Check sheet for the modelled part. Datum: model origin and axes. Units: mm. A direction names the side the tool comes from. Coordinates: 2 decimals unless noted, no trailing zeros. Loops run counter-clockwise (first coordinate to the right, second up) from the corner with the lowest first, then second, coordinate; pieces in that order, holes last. Notation, with made-up numbers: (69, 65.25) - (84, 65.25) arc R34 cw to (84, 96.25) - close; hole circle Ø8 at (70, -29.5). An arc over 180 degrees is marked (long way). Write each question's results on one line, items separated by ' | '. Start each with the question number.
1. Cross-section at B-B (z = 11). Record the cut outline in (x, y).
2. Tool access check on faces 4 (the face through (-2, 15, -31)), 5 (the face through (1, 46, -26)), 6 (the face through (-101, 32, 5)). Record the directions out of +Z, -Z, +X, -X, +Y, -Y that give a thin tool (end or side, any length) a straight path to the whole face; none if there is none.
3. Cross-section at C-C (y = 12). Record the cut outline in (x, z).
4. Draft check along X on faces 1 (the face through (-131, 5, 0)), 2 (the face through (20.24, 20.5, -26.07)), 3 (the face through (-41.17, 44.574, -26.07)). Enter one of: released by +X, released by -X, zero draft, split by the parting line, or undercut.
5. Cross-section at D-D (x = 26). Record the cut outline in (y, z).
6. Cross-section at A-A (x = 62). Record the cut outline in (y, z), and give its area (3 significant figures).
7. Gauge pin test, flat ends, axial feed: P1, Ø1.5, axis at x = -11.5, y = 48, coming from the +Z side; P2, Ø11, axis at y = 30.5, z = -26.5, coming from the -X side; P3, Ø11, axis at y = 29.5, z = -26.5, coming from the +X side. Record the tip position at first contact, or that the pin passes through.
8. Thickness scan on line 1 (Y direction, x = 37, z = 15); line 2 (X direction, y = 32, z = -24); line 3 (X direction, y = 55.5, z = -13). Record the ranges inside material, lowest first. Write a range as [from, to].
```python
from build123d import *

# Parameters (mm, degrees)
SKETCH_1_W          = 300
SKETCH_1_H          = 62
EXTRUDE_1_DEPTH     = 5
SKETCH_2_W          = 298.120909486
SKETCH_2_H          = 12
CUT_EXTRUDE_1_DEPTH = 1.5
SKETCH_3_W          = 15
SKETCH_3_H          = 62
SKETCH_3_W_2        = 14
CUT_EXTRUDE_2_DEPTH = 1.5
EXTRUDE_2_DEPTH     = 55
SKETCH_5_W          = 222
SKETCH_5_H          = 62
EXTRUDE_3_DEPTH     = 8
CUT_EXTRUDE_3_REACH = 174.708
SKETCH_6_W          = 41.333333333
SKETCH_6_H          = 27
SKETCH_6_W_2        = 41.333333334
FILLET_1_R          = 5


with BuildPart() as part:
    # 草图1 → 凸台-拉伸1 (new, symmetric)
    with BuildSketch(Plane(origin=(0, 0, 0), x_dir=(1, 0, 0), z_dir=(0, 1, 0))):
        Rectangle(SKETCH_1_W, SKETCH_1_H)
    extrude(amount=EXTRUDE_1_DEPTH, both=True)

    # 草图2 → 切除-拉伸1 (cut)
    with BuildSketch(Plane.XZ.offset(5)):
        with Locations((0.939545257, 25)):
            Rectangle(SKETCH_2_W, SKETCH_2_H)
    extrude(amount=-CUT_EXTRUDE_1_DEPTH, mode=Mode.SUBTRACT)

    # 草图3 → 切除-拉伸2 (cut)
    with BuildSketch(Plane.XZ.offset(5)):
        with Locations((-142.5, 0)):
            Rectangle(SKETCH_3_W, SKETCH_3_H)
        with Locations((143, 0)):
            Rectangle(SKETCH_3_W_2, SKETCH_3_H)
    extrude(amount=-CUT_EXTRUDE_2_DEPTH, mode=Mode.SUBTRACT)

    # 草图4 → 凸台-拉伸2 (add)
    with BuildSketch(Plane(origin=(0, 5, 0), x_dir=(1, 0, 0), z_dir=(0, 1, 0))):
        Polygon((-111, -31), (-111, 31), (111, 31), (111, -31), (103, -31), (103, 21), (-101, 21), (-101, -31), align=None)
    extrude(amount=EXTRUDE_2_DEPTH)

    # 草图5 → 凸台-拉伸3 (add)
    with BuildSketch(Plane(origin=(0, 60, 0), x_dir=(1, 0, 0), z_dir=(0, 1, 0))):
        Rectangle(SKETCH_5_W, SKETCH_5_H)
    extrude(amount=EXTRUDE_3_DEPTH)

    # 草图6 → 切除-拉伸3 (cut, up to next)
    with BuildSketch(Plane.XY.offset(-21), mode=Mode.PRIVATE) as cut_extrude_3_sk1:
        with Locations((-60.333333334, 32.5)):
            Rectangle(SKETCH_6_W, SKETCH_6_H)
    cut_extrude_3_tool1 = extrude(cut_extrude_3_sk1.sketch, amount=-CUT_EXTRUDE_3_REACH, mode=Mode.PRIVATE) & part.part
    # 草图6 → 切除-拉伸3 (cut, up to next)
    with BuildSketch(Plane.XY.offset(-21), mode=Mode.PRIVATE) as cut_extrude_3_sk2:
        with Locations((62.333333334, 32.5)):
            Rectangle(SKETCH_6_W, SKETCH_6_H)
    cut_extrude_3_tool2 = extrude(cut_extrude_3_sk2.sketch, amount=-CUT_EXTRUDE_3_REACH, mode=Mode.PRIVATE) & part.part
    # 草图6 → 切除-拉伸3 (cut, up to next)
    with BuildSketch(Plane.XY.offset(-21), mode=Mode.PRIVATE) as cut_extrude_3_sk3:
        with Locations((1, 32.5)):
            Rectangle(SKETCH_6_W_2, SKETCH_6_H)
    cut_extrude_3_tool3 = extrude(cut_extrude_3_sk3.sketch, amount=-CUT_EXTRUDE_3_REACH, mode=Mode.PRIVATE) & part.part
    add(cut_extrude_3_tool1.solids().sort_by_distance((-60.333333, 32.5, -21))[0], mode=Mode.SUBTRACT)
    add(cut_extrude_3_tool2.solids().sort_by_distance((62.333333, 32.5, -21))[0], mode=Mode.SUBTRACT)
    add(cut_extrude_3_tool3.solids().sort_by_distance((1, 32.5, -21))[0], mode=Mode.SUBTRACT)

    # 圆角1
    fillet_1_edges = [part.edges().sort_by_distance(p)[0] for p in [
        (-39.666666667, 46, -26),
        (-39.666666667, 19, -26),
        (-81, 19, -26),
        (-81, 46, -26),
        (83, 46, -26),
        (83, 19, -26),
        (41.666666667, 19, -26),
        (41.666666667, 46, -26),
        (21.666666667, 46, -26),
        (21.666666667, 19, -26),
        (-19.666666667, 19, -26),
        (-19.666666667, 46, -26),
    ]]
    fillet(fillet_1_edges, radius=FILLET_1_R)


solid = part.part
```
Established:
1) outline: (-150, -3.5) - (-135, -3.5) - (-135, -5) - (136, -5) - (136, -3.5) - (150, -3.5) - (150, 5) - (111, 5) - (111, 68) - (-111, 68) - (-111, 5) - (-150, 5) - close; hole (-101, 5) - (103, 5) - (103, 60) - (-101, 60) - close
2) face 4: -Z, +X, -X, +Y, -Y | face 5: +Z, -Z | face 6: +Z
3) outline: (-111, -31) - (111, -31) - (111, 31) - (103, 31) - (103, -21) - (-101, -21) - (-101, 31) - (-111, 31) - close
4) face 1: zero draft | face 2: undercut | face 3: undercut
5) outline: (-5, -31) - (68, -31) - (68, 31) - (60, 31) - (60, -21) - (5, -21) - (5, 31) - (-3.5, 31) - (-3.5, 19) - (-5, 19) - close
6) outline: (-5, -31) - (19, -31) - (19, -21) - (5, -21) - (5, 31) - (-3.5, 31) - (-3.5, 19) - (-5, 19) - close; (46, -31) - (68, -31) - (68, 31) - (60, 31) - (60, -21) - (46, -21) - close | area: 1,380 mm^2
7) P1: z = -21 | P2: x = -111 | P3: x = 111
8) line 1: [-5, 5], [60, 68] | line 2: [-111, -81], [-39.67, -19.67], [21.67, 41.67], [83, 111] | line 3: [-111, -101], [103, 111]
